Here's how the part is built. I have some questions about the finished solid (model axes, mm). Round coordinates to 2 decimals unless told otherwise and drop trailing zeros. Loops run counter-clockwise (first coordinate to the right, second up) from the corner with the lowest first, then second, coordinate; pieces in that order, holes last. Notation, with made-up numbers: M 44.25,-12 L 55.25,-12 A32 cw 55.25,21 Z; hole C -28,-13 d11. An arc over 180 degrees is marked long. Use a Markdown table: item, result.
from build123d import *

# Parameters (mm, degrees)
SKETCH1_R           = 40
BOSS_EXTRUDE1_DEPTH = 14
CHAMFER1_SIZE       = 8


with BuildPart() as part:
    # Sketch1 → Boss-Extrude1 (new body)
    with BuildSketch(Plane.XY):
        with BuildLine():
            Line((210, 170.2), (17.052877352, 187.727060846))
            ThreePointArc((17.052877352, 187.727060846), (-18.959205139, 187.54412425), (-54.27928922, 180.515951544))
            ThreePointArc((-54.27928922, 180.515951544), (-236.788094268, 105.291584642), (-400.963833305, -4.319071808))
            ThreePointArc((-400.963833305, -4.319071808), (-431.989523554, -114.33728667), (-339.549522969, -181.578995072))
            Line((-339.549522969, -181.578995072), (-3.863350797, -188.460405711))
            ThreePointArc((-3.863350797, -188.460405711), (6.604949005, -188.384247347), (17.052877352, -187.727060846))
            Line((17.052877352, -187.727060846), (210, -170.2))
            Line((210, -170.2), (210, 170.2))
        make_face()
        with Locations((-337.5, -81.6)):
            Circle(SKETCH1_R, mode=Mode.SUBTRACT)
    extrude(amount=BOSS_EXTRUDE1_DEPTH)

    # Chamfer1
    chamfer1_edges = [part.edges().sort_by_distance(p)[0] for p in [
        (-171.706436883, -185.019700391, 0),
        (-431.989523554, -114.33728667, 0),
        (-236.788094268, 105.291584642, 0),
        (-18.959205139, 187.54412425, 0),
        (113.526438676, 178.963530423, 0),
        (210, 0, 0),
        (113.526438676, -178.963530423, 0),
        (6.604949005, -188.384247347, 0),
    ]]
    chamfer(chamfer1_edges, length=CHAMFER1_SIZE)


solid = part.part
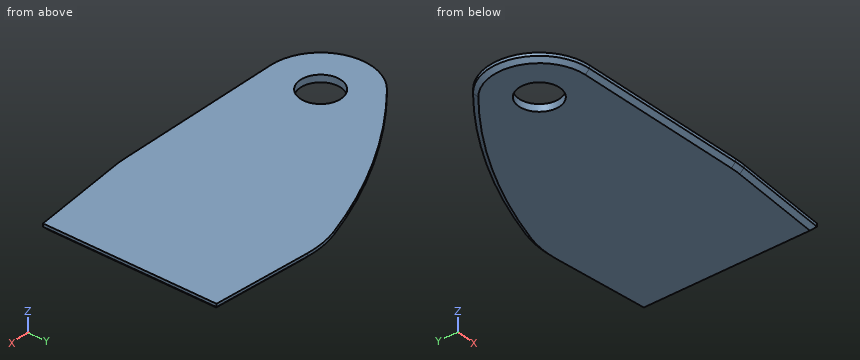
1. For pin 1 Ø6 at (x, z) = (-110, 7.5) entering from -Y; pin 2 Ø4 at (y, z) = (-133.5, 4) entering from -X; pin 3 Ø1 at (y, z) = (48, 6.5) entering from -X, each with a flat end and sliding along its axis, tell me the tip position at first contact or that it passes through.
Answer sheet:
| item | result |
|---|---|
| pin 1 | y = -186.35 |
| pin 2 | x = -420.93 |
| pin 3 | x = -329.76 |
2. Imagine slicing it at C-C, the plane x = 133. Write out the boundary of the cut face in (y, z).
Answer sheet:
| item | result |
|---|---|
| outline | M -177.19,8 L -169.16,0 L 169.16,0 L 177.19,8 L 177.19,14 L -177.19,14 Z |
3. Imagine slicing it at B-B, the plane z = 4.75. Write out the boundary of the cut face in (x, y), then the cut area to 3 significant figures.
Answer sheet:
| item | result |
|---|---|
| outline | M -398.9,-6.83 A96.75 ccw -339.48,-178.33 L -3.8,-185.21 A185.25 ccw 16.76,-184.49 L 206.75,-167.23 L 206.75,167.23 L 16.76,184.49 A185.25 ccw -53.34,177.4 A996.75 ccw Z; hole C -337.5,-81.6 d80 |
| area | 188,000 mm2 |
4. Imagine slicing it at A-A, the plane y = -81.6. Write out the boundary of the cut face in (x, z), then the cut area to 3 significant figures.
Answer sheet:
| item | result |
|---|---|
| outline | M -437.5,8 L -429.5,0 L -377.5,0 L -377.5,14 L -437.5,14 Z; M -297.5,0 L 202,0 L 210,8 L 210,14 L -297.5,14 Z |
| area | 7,880 mm2 |
5. I need wall thicknesses on probe 1 along Y at (x, z) = (-337.5, 3.75); probe 2 along Y at (x, z) = (-301, 9.5); probe 3 along Y at (x, z) = (-20.5, 4.5). Which ranges of each line are inside material? Lowest first, please. Write a range as from..to.
Answer sheet:
| item | result |
|---|---|
| probe 1 | -177.37..-121.6, -41.6..38.52 |
| probe 2 | -182.37..-97.96, -65.24..67.93 |
| probe 3 | -184.62..183.86 |
